CAD build for the part. Positions are in the model's coordinates, mm. A direction names the side the tool comes from. Give positions to 0.01 mm unless a question says otherwise; leave off trailing zeros. Write each loop counter-clockwise with the first axis right and the second up, starting at its lowest first coordinate (ties: lowest second). Pieces come first, ordered by that corner, then holes. Notation, with made-up numbers: M 19,-3.75 L 74,-3.75 A35 ccw 74,32.25 Z; hole C 30.5,34 d3. An arc over 180 degrees is marked long. One line per question, with ' | ' between items. Start each with the question number.
1. Cut at C-C, the plane y = 3.75. Write the cut outline in (x, z), then the cut area to 3 significant figures.
2. Which spindle directions (+Z, -Z, +X, -X, +Y, -Y) get a long thin tool onto all of the face, cutting with end or side? Do faces 4 (the face through (0, 9, 8)), 5 (the face through (-8, 9, 0)), 6 (the face through (0, 9, -8)). Say none if no direction does.
3. Cut at D-D, the plane z = -7.5. Count the separate pieces of the cut face and the enclosed holes in it, then the cut area to 3 significant figures.
4. Cut at B-B, the plane x = 0. Write the cut outline in (y, z), then the cut area to 3 significant figures.
5. Flat gauge pins, fed straight in: pin 1 (3.5 mm diameter, centred on y = 9, z = 15, fed in from +X); pin 2 (2.5 mm diameter, centred on x = 14.5, z = 2, fed in from +Y); pin 3 (11.5 mm diameter, centred on x = 0, z = 0, fed in from +Y); pin 4 (5 mm diameter, centred on y = 3, z = 9, fed in from +X). Where does each tip first touch, or does it go through?
6. Wall check: L1, parallel to X at y = 3.4, z = 0; L2, parallel to Y at x = -11, z = -10.5; L3, parallel to Z at x = 1, y = 4. Give the ranges that are in metal, low to high.
7. Pull direction Z, two halves, no side cores. Call faces 1 (the face through (15, 9, -4.5)), 2 (the face through (-11.87, 11.84, 11.69)), 3 (the face through (1, 6, 15)): released by +Z, released by -Z, zero draft, split by the parting line, or undercut.
8. Cut at A-A, the plane y = 6.75. Write the cut outline in (x, z).
```python
from build123d import *

# Parameters (mm, degrees)
SKETCH1_R                  = 17.5
SKETCH1_R_2                = 5
BOSS_EXTRUDE1_DEPTH        = 12
SKETCH4_R                  = 2.5
CUT_EXTRUDE2_DEPTH         = 28.504545079
SKETCH7_R                  = 4.5
CUT_EXTRUDE4_DEPTH         = 6
CUT_EXTRUDE5_DEPTH         = 6
CIRPATTERN1_COUNT          = 4
SKETCH9_W                  = 1.65
SKETCH9_H                  = 24.748737342
M4_TAPPED_HOLE1_AT_2_COUNT = 2
M4_TAPPED_HOLE1_AT_2_PITCH = 6
CHAMFER1_SIZE              = 1


with BuildPart() as part:
    # Sketch1 → Boss-Extrude1 (new body)
    with BuildSketch(Plane(origin=(0, 0, 0), x_dir=(1, 0, 0), z_dir=(0, 1, 0))):
        with Locations(Location((0, 0, 0), (0, 0, 270))):
            Circle(SKETCH1_R)
        with Locations(Location((0, 0, 0), (0, 0, 270))):
            Circle(SKETCH1_R_2, mode=Mode.SUBTRACT)
    extrude(amount=BOSS_EXTRUDE1_DEPTH)

    # Sketch4 → Cut-Extrude2 (cut, through all)
    with BuildSketch(Plane.XZ):
        with Locations(Location((0, 12.5, 0), (0, 0, 270))):
            Circle(SKETCH4_R)
        with Locations(Location((-12.5, 0, 0), (0, 0, 270))):
            Circle(SKETCH4_R)
        with Locations(Location((12.5, 0, 0), (0, 0, 270))):
            Circle(SKETCH4_R)
        with Locations(Location((0, -12.5, 0), (0, 0, 270))):
            Circle(SKETCH4_R)
    extrude(amount=-CUT_EXTRUDE2_DEPTH, mode=Mode.SUBTRACT)

    # Sketch7 → Cut-Extrude4 (cut)
    with BuildSketch(Plane(origin=(0, 12, 0), x_dir=(1, 0, 0), z_dir=(0, 1, 0))):
        with Locations(Location((0, 12.5, 0), (0, 0, 270))):
            Circle(SKETCH7_R)
        with Locations(Location((12.5, 0, 0), (0, 0, 270))):
            Circle(SKETCH7_R)
        with Locations(Location((0, -12.5, 0), (0, 0, 270))):
            Circle(SKETCH7_R)
        with Locations(Location((-12.5, 0, 0), (0, 0, 270))):
            Circle(SKETCH7_R)
    extrude(amount=-CUT_EXTRUDE4_DEPTH, mode=Mode.SUBTRACT)

    # Sketch8 → Cut-Extrude5 (cut)
    with BuildSketch(Plane(origin=(0, 12, 0), x_dir=(1, 0, 0), z_dir=(0, 1, 0))):
        with BuildLine():
            Line((-12.5, 4.5), (-21.528291401, 4.5))
            Line((-21.528291401, 4.5), (-21.528291401, -4.5))
            Line((-21.528291401, -4.5), (-12.5, -4.5))
            ThreePointArc((-12.5, -4.5), (-8, 0), (-12.5, 4.5))
        make_face()
    cut_extrude5 = extrude(amount=-CUT_EXTRUDE5_DEPTH, mode=Mode.SUBTRACT)

    # CirPattern1: Cut-Extrude5 ×4 about axis
    cirpattern1_axis = Axis((0, 0, 0), (0, 1, 0))
    for i in range(1, CIRPATTERN1_COUNT):
        add(cut_extrude5.rotate(cirpattern1_axis, i * 360 / CIRPATTERN1_COUNT), mode=Mode.SUBTRACT)

    # Sketch9 → M4 Tapped Hole1 (revolve, cut)
    with BuildSketch(Plane(origin=(0, 3, 0), x_dir=(0.7071067811865464, 0, -0.7071067811865488), z_dir=(0, 1, 0))):
        with Locations((0.825, 12.374368671)):
            Rectangle(SKETCH9_W, SKETCH9_H)
    m4_tapped_hole1 = revolve(axis=Axis((4.490128061, 3, 4.490128061), (-0.7071067811865487, 0, -0.7071067811865464)), mode=Mode.SUBTRACT)

    # M4 Tapped Hole1 at 2: M4 Tapped Hole1 ×2
    with Locations(*[(0, i * M4_TAPPED_HOLE1_AT_2_PITCH, 0) for i in range(1, M4_TAPPED_HOLE1_AT_2_COUNT)]):
        add(m4_tapped_hole1, mode=Mode.SUBTRACT)

    # Chamfer1
    chamfer1_edges = [part.edges().sort_by_distance(p)[0] for p in [
        (12.374368671, 12, 12.374368671),
        (-12.374368671, 12, 12.374368671),
        (-12.374368671, 12, -12.374368671),
        (12.374368671, 12, -12.374368671),
    ]]
    chamfer(chamfer1_edges, length=CHAMFER1_SIZE)


solid = part.part
```
Here are the results:
1) outline: M -13.37,-11.29 L -4.42,-2.34 A5 cw long -2.34,-4.42 L -11.29,-13.37 A17.5 ccw long Z; hole C -12.5,0 d5; hole C 0,-12.5 d5; hole C 0,12.5 d5; hole C 12.5,0 d5 | area: 768 mm^2
2) face 4: +Z, +Y | face 5: -X, +Y | face 6: -Z, +Y
3) separate pieces: 1 | enclosed holes: 2 | area: 354 mm^2
4) outline: M 0,-17.5 L 6,-17.5 L 6,-15 L 0,-15 Z; M 0,-10 L 6,-10 L 6,-8 L 12,-8 L 12,-5 L 0,-5 Z; M 0,5 L 12,5 L 12,8 L 6,8 L 6,10 L 0,10 Z; M 0,15 L 6,15 L 6,17.5 L 0,17.5 Z | area: 126 mm^2
5) pin 1: x = 11.43 | pin 2: y = 6 | pin 3: y = 12 | pin 4: x = 16.25
6) L1: -17.5 to -15, -10 to -5, 5 to 10, 15 to 17.5 | L2: 0 to 1.39, 4.61 to 7.39, 10.61 to 12 | L3: -17.47 to -14.79, -10.21 to -4.9, 4.9 to 10.21, 14.79 to 17.47
7) face 1: undercut | face 2: released by +Z | face 3: zero draft
8) outline: M -16.91,-4.5 A17.5 ccw -4.5,-16.91 L -4.5,-12.5 A4.5 cw 4.5,-12.5 L 4.5,-16.91 A17.5 ccw 16.91,-4.5 L 12.5,-4.5 A4.5 cw 12.5,4.5 L 16.91,4.5 A17.5 ccw 4.5,16.91 L 4.5,12.5 A4.5 cw -4.5,12.5 L -4.5,16.91 A17.5 ccw -16.91,4.5 L -12.5,4.5 A4.5 cw -12.5,-4.5 Z; hole C 0,0 d10
